from build123d import *

# Parameters (mm, degrees)
SKETCH_1_R          = 7
EXTRUDE_1_DEPTH     = 3
SKETCH_2_R          = 4
EXTRUDE_2_DEPTH     = 10.5
SKETCH_3_R          = 3
EXTRUDE_3_DEPTH     = 8
SKETCH_4_R          = 3
SKETCH_4_R_2        = 2.25
CUT_EXTRUDE_1_DEPTH = 0.8
FILLET_1_R          = 2
SKETCH_5_W          = 17.035496118
SKETCH_5_H          = 1.5
CUT_EXTRUDE_2_DEPTH = 1.5
CHAMFER_1_SIZE      = 0.3


with BuildPart() as part:
    # 草图1 → 凸台-拉伸1 (new body)
    with BuildSketch(Plane.XY):
        Circle(SKETCH_1_R)
    extrude(amount=EXTRUDE_1_DEPTH)

    # 草图2 → 凸台-拉伸2 (add)
    with BuildSketch(Plane.XY.offset(3)):
        with Locations(Location((0, 0, 0), (0, 0, 180))):
            Circle(SKETCH_2_R)
    extrude(amount=EXTRUDE_2_DEPTH)

    # 草图3 → 凸台-拉伸3 (add)
    with BuildSketch(Plane.XY.offset(13.5)):
        Circle(SKETCH_3_R)
    extrude(amount=EXTRUDE_3_DEPTH)

    # 草图4 → 切除-拉伸1 (cut)
    with BuildSketch(Plane.XY.offset(13.5)):
        Circle(SKETCH_4_R)
        Circle(SKETCH_4_R_2, mode=Mode.SUBTRACT)
    extrude(amount=CUT_EXTRUDE_1_DEPTH, mode=Mode.SUBTRACT)

    # 圆角1
    fillet_1_edges = [part.edges().sort_by_distance(p)[0] for p in [
        (-7, 0, 0),
    ]]
    fillet(fillet_1_edges, radius=FILLET_1_R)

    # 草图5 → 切除-拉伸2 (cut)
    with BuildSketch(Plane(origin=(0, 0, 0), x_dir=(-1, 0, 0), z_dir=(0, 0, -1))):
        Rectangle(SKETCH_5_W, SKETCH_5_H)
    extrude(amount=-CUT_EXTRUDE_2_DEPTH, mode=Mode.SUBTRACT)

    # 倒角1
    chamfer_1_edges = [part.edges().sort_by_distance(p)[0] for p in [
        (-3, 0, 21.5),
        (4, 0, 13.5),
    ]]
    chamfer(chamfer_1_edges, length=CHAMFER_1_SIZE)


solid = part.part
For this review, take the finished solid that the model builds, in its own axes (mm). A direction names the side the tool comes from. Give positions to 0.01 mm unless a question says otherwise; leave off trailing zeros. Loops run counter-clockwise (first coordinate to the right, second up) from the corner with the lowest first, then second, coordinate; pieces in that order, holes last. Notation, with made-up numbers: (63, -31) - (110, -31) arc R18 cw to (110, -10) - close; hole circle Ø3 at (-28, 25.5). An arc over 180 degrees is marked (long way). Write each question's results on one line, items separated by ' | '.
(1) Take a section at B-B (x = 0). Give the boundary of the cut face in (y, z), then the cut area to 3 significant figures.
Conclusion:
outline: (-7, 2) arc R2 ccw to (-5, 0) - (-0.75, 0) - (-0.75, 1.5) - (0.75, 1.5) - (0.75, 0) - (5, 0) arc R2 ccw to (7, 2) - (7, 3) - (4, 3) - (4, 13.2) - (3.7, 13.5) - (2.25, 13.5) - (2.25, 14.3) - (3, 14.3) - (3, 21.2) - (2.7, 21.5) - (-2.7, 21.5) - (-3, 21.2) - (-3, 14.3) - (-2.25, 14.3) - (-2.25, 13.5) - (-3.7, 13.5) - (-4, 13.2) - (-4, 3) - (-7, 3) - close | area: 169 mm^2
(2) Draft analysis for pull direction Y (two halves, no side actions). For faces 4 (the cylindrical face through (-3, 0, 18)), 5 (the flat face through (0, -0.75, 1)), 6 (the flat face through (0, 0.75, 1)), 7 (the flat face through (3, -3, 3)), state which applies: +Y half, -Y half, draft (parallel to the pull), parting line (faces both ways), or undercut.
Conclusion:
face 4: parting line | face 5: undercut | face 6: undercut | face 7: draft
(3) Take a section at C-C (z = 17.75). Give the boundary of the cut face in (x, y), then the cut area to 3 significant figures.
Conclusion:
outline: circle Ø6 at (0, 0) | area: 28.3 mm^2
(4) For pin 1 Ø1 at (x, z) = (-3, 3) entering from +Y; pin 2 Ø1.7 at (x, z) = (-1, 1) entering from +Y; pin 3 Ø5 at (x, y) = (3, -5.5) entering from +Z (3 decimals), all flat-tipped, find the tip position at first contact; note any pin that passes through.
Conclusion:
pin 1: y = 6.54 | pin 2: y = 6.96 | pin 3: z = 13.435
(5) For faces 1 (the flat face through (0, 0, 1.5)), 2 (the flat face through (-2, 2, 13.5)), 3 (the cylindrical face through (0.867, 3.905, 8.029)), list the 3-axis set-ups (+Z, -Z, +X, -X, +Y, -Y) from which the entire face can be reached by the end or side of a thin tool; tool diameter is ignored.
Conclusion:
face 1: -Z, +X, -X | face 2: none | face 3: +Z
(6) Take a section at A-A (y = 0). Give the boundary of the cut face in (x, z).
Conclusion:
outline: (-7, 2) arc R2 ccw to (-6.94, 1.5) - (6.94, 1.5) arc R2 ccw to (7, 2) - (7, 3) - (4, 3) - (4, 13.2) - (3.7, 13.5) - (2.25, 13.5) - (2.25, 14.3) - (3, 14.3) - (3, 21.2) - (2.7, 21.5) - (-2.7, 21.5) - (-3, 21.2) - (-3, 14.3) - (-2.25, 14.3) - (-2.25, 13.5) - (-3.7, 13.5) - (-4, 13.2) - (-4, 3) - (-7, 3) - close
(7) For line 1 along Z through (x, y) = (2.5, -1.5); line 2 along Z through (x, y) = (-4, -0.5); line 3 along Z through (x, y) = (-4, 1.5), list the stretches that pass through material, from the lowest coordinate up.
Conclusion:
line 1: 0 to 13.5, 14.3 to 21.28 | line 2: 1.5 to 3 | line 3: 0 to 3
(8) Take a section at D-D (z = 14). Give the boundary of the cut face in (x, y).
Conclusion:
outline: circle Ø4.5 at (0, 0)
